```python
from build123d import *

# Parameters (mm, degrees)
BOSS_EXTRUDE1_DEPTH = 6
SKETCH2_W           = 6
SKETCH2_H           = 59.975118876
CUT_EXTRUDE1_DEPTH  = 6


with BuildPart() as part:
    # Sketch1 → Boss-Extrude1 (new body)
    with BuildSketch(Plane.XY):
        Polygon((107.036449202, -34.108774603), (102.587015051, 90.196105325), (122.563832413, 90.911166016), (122.850005344, 82.916286089), (147.788760974, 83.808957004), (147.502588043, 91.803836932), (167.479405405, 92.518897623), (171.928839556, -31.785982304), (152.013983639, -32.498825115), (152.013983639, -24.108777743), (127.013266564, -24.108777743), (127.013266564, -33.393713911), align=None)
    extrude(amount=BOSS_EXTRUDE1_DEPTH)

    # Sketch2 → Cut-Extrude1 (cut)
    with BuildSketch(Plane.XY.offset(6)):
        with Locations((139.513625101, 53.898004923)):
            Rectangle(SKETCH2_W, SKETCH2_H)
    extrude(amount=-CUT_EXTRUDE1_DEPTH, mode=Mode.SUBTRACT)


solid = part.part
```
Here's how the part is built. I have some questions about the finished solid (model axes, mm). A direction names the side the tool comes from. Give positions to 0.01 mm unless a question says otherwise; leave off trailing zeros. Loops run counter-clockwise (first coordinate to the right, second up) from the corner with the lowest first, then second, coordinate; pieces in that order, holes last. Notation, with made-up numbers: (72.5, -3) -> (102.5, -3) arc R21 cw to (102.5, 16) -> close; hole circle Ø7 at (42.5, 52.5). An arc over 180 degrees is marked (long way). Use one line per item in the form item = value. Start each with the question number.
1) Thinking about a two-plate mould opening in X: for faces 4 (the face through (130, 30, 0)), 5 (the face through (152.014, -28, 3)), 6 (the face through (127.013, -29, 3)), which applies, +X half, -X half, draft (parallel to the pull), parting line (faces both ways), or undercut?
2) Which directions (+Z, -Z, +X, -X, +Y, -Y) give clear straight access to the entire face, cutting with the end or side of a thin tool? Please do faces 1 (the face through (142.514, 53, 3)), 2 (the face through (130, 30, 6)), 3 (the face through (140, -24.109, 3)).
3) For P1, Ø1, axis at y = 2, z = 2, coming from the +X side; P2, Ø3, axis at y = -28, z = 2.5, coming from the +X side; P3, Ø1.8, axis at y = -26, z = 4, coming from the -X side, each with a flat end and sliding along its axis, tell me the tip position at first contact or that it passes through.
4) Imagine slicing it at B-B (z = 1.25). Please give me the cut outline in (x, y).
5) Imagine slicing it at A-A (y = 38.5). Please give me the cut outline in (x, z).
6) Imagine slicing it at D-D (y = 13). Please give me the cut outline in (x, z), then the cut area to 3 significant figures.
7) Please list where these lines run through material, in increasing order: line 1 along X through (y, z) = (62, 2.5); line 2 along X through (y, z) = (85, 3); line 3 along X through (y, z) = (-8.5, 2.9).
8) Imagine slicing it at C-C (x = 144). Please give me the cut outline in (y, z), then the cut area to 3 significant figures.
Check values:
q1.face_4 = draft
q1.face_5 = undercut
q1.face_6 = undercut
q2.face_1 = +Z, -Z, +Y
q2.face_2 = +Z, +X, -X, +Y, -Y
q2.face_3 = +Z, -Z, -Y
q3.P1 = 170.74
q3.P2 = 171.85
q3.P3 = 106.71
q4.outline = (102.59, 90.2) -> (107.04, -34.11) -> (127.01, -33.39) -> (127.01, -24.11) -> (152.01, -24.11) -> (152.01, -32.5) -> (171.93, -31.79) -> (167.48, 92.52) -> (147.5, 91.8) -> (147.79, 83.81) -> (142.51, 83.62) -> (142.51, 23.91) -> (136.51, 23.91) -> (136.51, 83.41) -> (122.85, 82.92) -> (122.56, 90.91) -> close
q5.outline = (104.44, 0) -> (136.51, 0) -> (136.51, 6) -> (104.44, 6) -> close; (142.51, 0) -> (169.41, 0) -> (169.41, 6) -> (142.51, 6) -> close
q6.outline = (105.35, 0) -> (170.33, 0) -> (170.33, 6) -> (105.35, 6) -> close
q6.area = 390 mm^2
q7.line_1 = 103.6 to 136.51, 142.51 to 168.57
q7.line_2 = 102.77 to 122.78, 147.75 to 167.75
q7.line_3 = 106.12 to 171.1
q8.outline = (-24.11, 0) -> (83.67, 0) -> (83.67, 6) -> (-24.11, 6) -> close
q8.area = 647 mm^2
